Part model, mm, in its own coordinate system. Face numbers are marked on the shaded views. Give positions to 0.01 mm unless a question says otherwise; leave off trailing zeros. Order: outer loops, then holes, each group sorted by start corner. A loop starts at its lowest first (then second) coordinate and runs counter-clockwise, first axis right, second up. Notation, with made-up numbers: M 25.5,33.25 L 43.5,33.25 A14 ccw 43.5,44.25 Z; hole C -12.5,20 d3. An arc over 180 degrees is marked long. Answer as a JSON object with one key per item and string values.
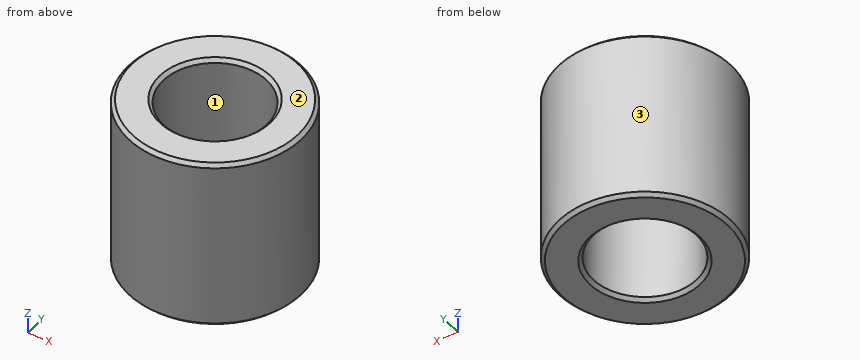
from build123d import *

# Parameters (mm, degrees)
SKETCH1_R           = 25
SKETCH1_R_2         = 15
BOSS_EXTRUDE1_DEPTH = 50
CHAMFER1_SIZE       = 1


with BuildPart() as part:
    # Sketch1 → Boss-Extrude1 (new body)
    with BuildSketch(Plane.XY):
        Circle(SKETCH1_R)
        Circle(SKETCH1_R_2, mode=Mode.SUBTRACT)
    extrude(amount=BOSS_EXTRUDE1_DEPTH)

    # Chamfer1
    chamfer1_edges = [part.edges().sort_by_distance(p)[0] for p in [
        (-25, 0, 0),
        (-25, 0, 50),
        (-15, 0, 0),
        (-15, 0, 50),
    ]]
    chamfer(chamfer1_edges, length=CHAMFER1_SIZE)


solid = part.part
1. Probe line 1 along X through (y, z) = (-6, 9.5); line 2 along Y through (x, z) = (-7, 9); line 3 along Y through (x, z) = (-1.5, 26.5). List the from-to ranges inside material, lowest first.
Worked answers:
{"line 1": "x = -24.27 to -13.75, 13.75 to 24.27", "line 2": "y = -24 to -13.27, 13.27 to 24", "line 3": "y = -24.95 to -14.92, 14.92 to 24.95"}
2. Pin check, flat tips, straight feed: P1, Ø8, axis at x = -7, z = 12, coming from the -Y side; P2, Ø2, axis at y = -20, z = 41.5, coming from the +X side; P3, Ø2, axis at y = 15, z = 36.5, coming from the -X side. Stop position of each tip, or through.
Worked answers:
{"P1": "stops at y = -24.82", "P2": "stops at x = 16.25", "P3": "stops at x = -20.71"}
3. Two-plate mould, pull along X, no slides. Class the marked faces 1, 2 and 3: +X half, -X half, draft (parallel to the pull), parting line (faces both ways), or undercut.
Worked answers:
{"face 1": "undercut", "face 2": "draft", "face 3": "parting line"}
4. Cut at C-C on z = 25.5. Give the cut face in (x, y).
Worked answers:
{"outline": "C 0,0 d50; hole C 0,0 d30"}
5. Cut at A-A on y = 0. Give the cut face in (x, z).
Worked answers:
{"outline": "M -25,1 L -24,0 L -16,0 L -15,1 L -15,49 L -16,50 L -24,50 L -25,49 Z; M 15,1 L 16,0 L 24,0 L 25,1 L 25,49 L 24,50 L 16,50 L 15,49 Z"}
